Here's how the part is built. I have some questions about the finished solid (model axes, mm). A direction names the side the tool comes from. Coordinates: 2 decimals unless noted, no trailing zeros. Order: outer loops, then holes, each group sorted by start corner. A loop starts at its lowest first (then second) coordinate and runs counter-clockwise, first axis right, second up. Notation, with made-up numbers: (19.25, -4.5) -> (38.25, -4.5) arc R21 ccw to (38.25, 3.5) -> close; hole circle Ø2 at (-31, -26.5). An arc over 180 degrees is marked (long way). One line per item, written item: value. Start each with the question number.
```python
from build123d import *

# Parameters (mm, degrees)
FRAME_BODY_200_DEPTH        = 100
CENTRE_RECESS_SKETCH_W      = 160
CENTRE_RECESS_SKETCH_H      = 60
CENTRE_RECESS_CUT_DEPTH     = 150
WINDOW_A_CUT_REACH          = 246.949
WINDOW_A_SKETCH_80X60_W     = 160
WINDOW_A_SKETCH_80X60_H     = 60
WINDOW_B_CUT_REACH          = 239.487
WINDOW_B_SKETCH_W           = 160
WINDOW_B_SKETCH_H           = 80
WINDOW_CORNER_FILLETS_R10_R = 10
ANCHOR_BOSS_SKETCH_90_R     = 45
ANCHOR_BOSS_90_DEPTH        = 20
ANCHOR_BORE_SKETCH_50_R     = 25
ANCHOR_BORE_50_DEPTH        = 245.948974278


with BuildPart() as part:
    # Frame Profile Sketch → Frame Body 200 (new, symmetric)
    with BuildSketch(Plane(origin=(0, 0, 0), x_dir=(0, 0, -1), z_dir=(1, 0, 0))):
        Polygon((200, 0), (170, 100), (80, 100), (0, 0), align=None)
        Polygon((155.119386982, 80), (89.61249695, 80), (41.61249695, 20), (173.119386982, 20), align=None, mode=Mode.SUBTRACT)
    extrude(amount=FRAME_BODY_200_DEPTH, both=True)

    # Centre Recess Sketch → Centre Recess Cut (cut)
    with BuildSketch(Plane.XY):
        with Locations((0, 50)):
            Rectangle(CENTRE_RECESS_SKETCH_W, CENTRE_RECESS_SKETCH_H)
    extrude(amount=-CENTRE_RECESS_CUT_DEPTH, mode=Mode.SUBTRACT)

    # Window A Sketch 80x60 → Window A Cut (cut, up to next)
    with BuildSketch(Plane(origin=(0, 100, 0), x_dir=(1, 0, 0), z_dir=(0, 1, 0)), mode=Mode.PRIVATE) as window_a_cut_sk1:
        with Locations((0, 90)):
            Rectangle(WINDOW_A_SKETCH_80X60_W, WINDOW_A_SKETCH_80X60_H)
    window_a_cut_tool1 = extrude(window_a_cut_sk1.sketch, amount=-WINDOW_A_CUT_REACH, mode=Mode.PRIVATE) & part.part
    add(window_a_cut_tool1.solids().sort_by_distance((0, 100, -90))[0], mode=Mode.SUBTRACT)

    # Window B Sketch → Window B Cut (cut, up to next)
    with BuildSketch(Plane(origin=(0, 20, 0), x_dir=(1, 0, 0), z_dir=(0, 1, 0)), mode=Mode.PRIVATE) as window_b_cut_sk1:
        with Locations((0, 40)):
            Rectangle(WINDOW_B_SKETCH_W, WINDOW_B_SKETCH_H)
    window_b_cut_tool1 = extrude(window_b_cut_sk1.sketch, amount=-WINDOW_B_CUT_REACH, mode=Mode.PRIVATE) & part.part
    add(window_b_cut_tool1.solids().sort_by_distance((0, 20, -40))[0], mode=Mode.SUBTRACT)

    # Window Corner Fillets R10
    window_corner_fillets_r10_edges = [part.edges().sort_by_distance(p)[0] for p in [
        (80, 90, -120),
        (-80, 90, -120),
        (-80, 10, -80),
        (80, 10, -80),
    ]]
    fillet(window_corner_fillets_r10_edges, radius=WINDOW_CORNER_FILLETS_R10_R)

    # Anchor Boss Sketch Ø90 → Anchor Boss Ø90 (add)
    with BuildSketch(Plane(origin=(0, 100, 0), x_dir=(1, 0, 0), z_dir=(0, 1, 0))):
        with Locations((0, 120)):
            Circle(ANCHOR_BOSS_SKETCH_90_R)
    extrude(amount=-ANCHOR_BOSS_90_DEPTH)

    # Anchor Bore Sketch Ø50 → Anchor Bore Ø50 (cut, through all)
    with BuildSketch(Plane(origin=(0, 100, 0), x_dir=(1, 0, 0), z_dir=(0, 1, 0))):
        with Locations(Location((0, 120, 0), (0, 0, 270))):
            Circle(ANCHOR_BORE_SKETCH_50_R)
    extrude(amount=-ANCHOR_BORE_50_DEPTH, mode=Mode.SUBTRACT)


solid = part.part
```
Q1. Imagine slicing it at B-B (x = 0). Write out the boundary of the cut face in (y, z), plus the area to 3 significant figures.
Q2. Imagine slicing it at C-C (y = 8). Write out the boundary of the cut face in (x, z).
Q3. I need wall thicknesses on line 1 (Y direction, x = -35, z = -105); line 2 (X direction, y = 90, z = -86); line 3 (X direction, y = 43.5, z = -46). Which ranges of each line are inside material? Lowest first, please.
Q4. If we mould it in two halves opening along Y, with no side actions, what happens to faces 4 (the face through (24, 20, -136)), 5 (the face through (90.14, 50.7, -40.56)), 6 (the face through (24, 0, -143)), 7 (the face through (-76.99, 9.86, -77.15))? For each: +Y half, -Y half, draft (parallel to the pull), parting line (faces both ways), or undercut.
Q5. For P1, Ø10, axis at x = -52, y = 86, coming from the +Z side; P2, Ø1.5, axis at x = 78, y = 85.5, coming from the +Z side; P3, Ø2, axis at x = -11, y = 72.5, coming from the -Z side, each with a flat end and sliding along its axis, tell me the tip position at first contact or that it passes through.
Q6. For faces 1 (the face through (-76.99, 89.86, -117.15)), 2 (the face through (77.15, 9.86, -76.99)), 3 (the face through (-89.86, 50.42, -65.95)), which set-ups out of +Z, -Z, +X, -X, +Y, -Y let a thin tool reach every point of the face, with its end or its side?
Q7. Imagine slicing it at A-A (z = -25). Write out the boundary of the cut face in (x, y).
Q8. Imagine slicing it at D-D (x = -36). Write out the boundary of the cut face in (y, z).
Completed:
1. outline: (0, -200) -> (100, -170) -> (100, -145) -> (80, -145) -> (80, -155.12) -> (20, -173.12) -> (20, -145) -> (0, -145) -> close; (0, -95) -> (20, -95) -> (20, -80) -> (0, -80) -> close; (80, -95) -> (100, -95) -> (100, -75) -> (80, -75) -> close
1. area: 3,550 mm2
2. outline: (-100, -197.6) -> (100, -197.6) -> (100, -6.4) -> (80, -6.4) -> (80, -70) arc R10 cw to (70, -80) -> (-70, -80) arc R10 cw to (-80, -70) -> (-80, -6.4) -> (-100, -6.4) -> close; hole circle Ø50 at (0, -120)
3. line 1: y = 0 to 20, 80 to 100
3. line 2: x = -100 to -80, -29.48 to 29.48, 80 to 100
3. line 3: x = -100 to -80, 80 to 100
4. face 4: undercut
4. face 5: +Y half
4. face 6: -Y half
4. face 7: draft
5. P1: stops at z = -120
5. P2: stops at z = -114.84
5. P3: stops at z = -178.55
6. face 1: +Z, +Y
6. face 2: +Z, +Y, -Y
6. face 3: +X, -X
7. outline: (-100, 0) -> (-80, 0) -> (-80, 31.25) -> (-100, 31.25) -> close; (80, 0) -> (100, 0) -> (100, 31.25) -> (80, 31.25) -> close
8. outline: (0, -200) -> (100, -170) -> (100, -93) -> (80, -93) -> (80, -155.12) -> (20, -173.12) -> (20, -80) -> (0, -80) -> close
